```python
from build123d import *

# Parameters (mm, degrees)
CROSS_HOLE_3_DEPTH      = 125.080618954
CROSS_HOLE_3_DEPTH_BACK = 125.080618954
CROSS_HOLE_SKETCH_R     = 1.5
CHAMFER_2X45_SIZE       = 2


with BuildPart() as part:
    # Pin Profile Sketch → Pin Body (revolve)
    with BuildSketch(Plane.XY, mode=Mode.PRIVATE) as pin_body_sk:
        Polygon((0, -7.5), (112, -7.5), (112, -16), (122, -16), (122, 0), (0, 0), align=None)
    revolve(pin_body_sk.sketch.rotate(Axis((122, 0, 0), (-1, 0, 0)), 180), axis=Axis((122, 0, 0), (-1, 0, 0)))

    # Cross Hole Sketch → Cross Hole Ø3 (cut, two sides: drawn at the far end of the back side and taken through both)
    with BuildSketch(Plane.XY.offset(-CROSS_HOLE_3_DEPTH_BACK)):
        with Locations((7, 0)):
            Circle(CROSS_HOLE_SKETCH_R)
    extrude(amount=CROSS_HOLE_3_DEPTH + CROSS_HOLE_3_DEPTH_BACK, mode=Mode.SUBTRACT)

    # Chamfer 2x45°
    chamfer_2x45_edges = [part.edges().sort_by_distance(p)[0] for p in [
        (122, -16, 0),
        (0, -7.5, 0),
    ]]
    chamfer(chamfer_2x45_edges, length=CHAMFER_2X45_SIZE)


solid = part.part
```
Could you check a few things on this model? Use its own coordinates, in mm. A direction names the side the tool comes from. Give positions to 0.01 mm unless a question says otherwise; leave off trailing zeros. Loops run counter-clockwise (first coordinate to the right, second up) from the corner with the lowest first, then second, coordinate; pieces in that order, holes last. Notation, with made-up numbers: (-29.75, 27) - (-6.75, 27) arc R24 cw to (-6.75, 66) - close; hole circle Ø7 at (34, 66). An arc over 180 degrees is marked (long way). Answer in a Markdown table with one row per item. Add a question column.
Q1. For pin 1 (6 mm diameter, centred on x = 23, z = 3.5, fed in from +Y); pin 2 (1 mm diameter, centred on x = 13.5, y = -1.5, fed in from +Z); pin 3 (1 mm diameter, centred on x = 63.5, y = 0.5, fed in from +Z), each with a flat end and sliding along its axis, tell me the tip position at first contact or that it passes through.
Q2. If we section it at C-C (x = 7): List the corners of the cut face in (y, z) for me.
Q3. If we section it at A-A (y = 0): List the corners of the cut face in (x, z) for me.
Q4. Please list where these lines run through material, in increasing order: L1, parallel to X at y = 0, z = 1.5; L2, parallel to Y at x = 7, z = 0.5; L3, parallel to X at y = 10, z = 6. Write a range as from..to.
Q5. We'd pull the mould along X, two halves only. Please class faces 1 (the face through (5.5, 0.07, -0.11)), 2 (the face through (116.06, -3.47, 15.62)), 3 (the face through (122, 0, 0)), 4 (the face through (112, -6.89, 3.33)): +X half, -X half, draft (parallel to the pull), parting line (faces both ways), or undercut.
Q6. If we section it at B-B (z = 0): List the corners of the cut face in (x, y) for me.
Q7. If we section it at D-D (x = 102): List the corners of the cut face in (y, z) for me.
Q8. Which directions (+Z, -Z, +X, -X, +Y, -Y) give clear straight access to the entire face, cutting with the end or side of a thin tool? Please do faces 5 (the face through (0, 0, 0)), 6 (the face through (57.77, 4.032, -6.324)).
The answers:
| question | item | result |
|---|---|---|
| 1 | pin 1 | stops at y = 7.48 |
| 1 | pin 2 | stops at z = 7.43 |
| 1 | pin 3 | stops at z = 7.5 |
| 2 | outline | (-1.5, -7.35) - (-1.5, 7.35) arc R7.5 ccw to start; (1.5, -7.35) arc R7.5 ccw to (1.5, 7.35) - close |
| 3 | outline | (0, -5.5) - (2, -7.5) - (5.5, -7.5) - (5.5, 7.5) - (2, 7.5) - (0, 5.5) - close; (8.5, -7.5) - (112, -7.5) - (112, -16) - (120, -16) - (122, -14) - (122, 14) - (120, 16) - (112, 16) - (112, 7.5) - (8.5, 7.5) - close |
| 4 | L1 | x = 0..5.5, 8.5..122 |
| 4 | L2 | y = -7.48..-1.5, 1.5..7.48 |
| 4 | L3 | x = 112..122 |
| 5 | face 1 | undercut |
| 5 | face 2 | draft |
| 5 | face 3 | +X half |
| 5 | face 4 | -X half |
| 6 | outline | (0, -5.5) - (2, -7.5) - (112, -7.5) - (112, -16) - (120, -16) - (122, -14) - (122, 14) - (120, 16) - (112, 16) - (112, 7.5) - (2, 7.5) - (0, 5.5) - close; hole circle Ø3 at (7, 0) |
| 7 | outline | circle Ø15 at (0, 0) |
| 8 | face 5 | +Z, -Z, -X, +Y, -Y |
| 8 | face 6 | -X |
